```python
from build123d import *

# Parameters (mm, degrees)
BOSS_EXTRUDE1_DEPTH = 7
CHAMFER1_SIZE       = 20


with BuildPart() as part:
    # Sketch1 → Boss-Extrude1 (new, symmetric)
    with BuildSketch(Plane.XY):
        Polygon((0, 0), (192, 0), (192, 20), (20, 70), (0, 70), align=None)
    extrude(amount=BOSS_EXTRUDE1_DEPTH, both=True)

    # Chamfer1
    chamfer1_edges = [part.edges().sort_by_distance(p)[0] for p in [
        (0, 0, 0),
    ]]
    chamfer(chamfer1_edges, length=CHAMFER1_SIZE)


solid = part.part
```
Verification items for the finished model (mm, model axes). Give positions to 0.01 mm unless a question says otherwise; leave off trailing zeros. Loops run counter-clockwise (first coordinate to the right, second up) from the corner with the lowest first, then second, coordinate; pieces in that order, holes last.
1. Section check B-B, the plane y = 53.5. Enter the section's corners in (x, z), then the cut area to 3 significant figures.
2. Section check A-A, the plane z = 3.75. Enter the section's corners in (x, y), then the cut area to 3 significant figures.
3. Thickness scan on line 1 (X direction, y = 11, z = -0.25); line 2 (Y direction, x = 91, z = 4.25); line 3 (X direction, y = 7.5, z = 5.75). Record the ranges inside material, lowest first.
4. Go/stop test with flat-tipped pins: pin 1 Ø1 at (x, z) = (103, -4) entering from +Y; pin 2 Ø1 at (x, z) = (34, 3.5) entering from +Y. Record where each tip stops, or that it passes through.
5. Section check C-C, the plane x = 164.5. Enter the section's corners in (y, z).
Geometry says:
1. outline: (0, -7) - (76.76, -7) - (76.76, 7) - (0, 7) - close
1. area: 1,070 mm2
2. outline: (0, 20) - (20, 0) - (192, 0) - (192, 20) - (20, 70) - (0, 70) - close
2. area: 8,940 mm2
3. line 1: x = 9 to 192
3. line 2: y = 0 to 49.36
3. line 3: x = 12.5 to 192
4. pin 1: stops at y = 46.02
4. pin 2: stops at y = 66.08
5. outline: (0, -7) - (27.99, -7) - (27.99, 7) - (0, 7) - close
